Work out the finished part from the listing and answer in its coordinate system (mm). Face numbers are marked on the shaded views. Coordinates: 2 decimals unless noted, no trailing zeros. Loops run counter-clockwise (first coordinate to the right, second up) from the corner with the lowest first, then second, coordinate; pieces in that order, holes last.
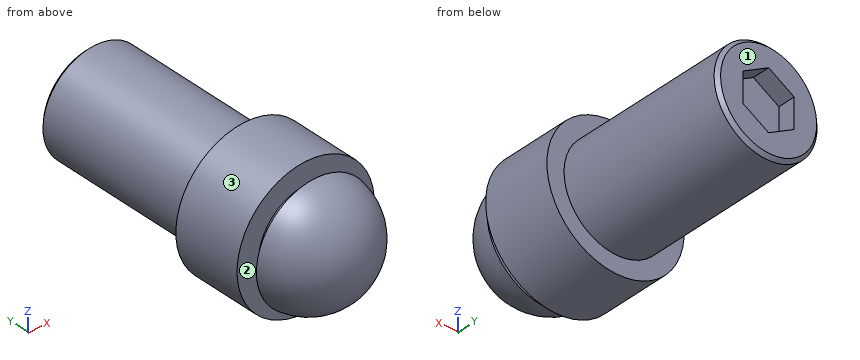
```python
from build123d import *

# Parameters (mm, degrees)
SKETCH1_R           = 1.5
BOSS_EXTRUDE1_DEPTH = 5
SKETCH2_R           = 2
BOSS_EXTRUDE2_DEPTH = 2
CUT_EXTRUDE1_DEPTH  = 0.5
CHAMFER1_SIZE       = 0.1


with BuildPart() as part:
    # Sketch1 → Boss-Extrude1 (new body)
    with BuildSketch(Plane(origin=(0, 0, 0), x_dir=(1, 0, 0), z_dir=(0, 1, 0))):
        with Locations(Location((0, 0, 0), (0, 0, 270))):
            Circle(SKETCH1_R)
    extrude(amount=BOSS_EXTRUDE1_DEPTH)

    # Sketch2 → Boss-Extrude2 (add)
    with BuildSketch(Plane.XZ):
        with Locations(Location((0, 0, 0), (0, 0, 270))):
            Circle(SKETCH2_R)
    extrude(amount=BOSS_EXTRUDE2_DEPTH)

    # Sketch3 → Revolve1 (revolve)
    with BuildSketch(Plane.XY):
        with BuildLine():
            Line((0, -2), (0, -3.798690772))
            ThreePointArc((0, -3.798690772), (1.135010023, -3.368611599), (1.7, -2.294366668))
            Line((1.7, -2.294366668), (1.376675655, -2.294366668))
            Line((1.376675655, -2.294366668), (1.376675655, -2))
            Line((1.376675655, -2), (0, -2))
        make_face()
    revolve(axis=Axis((0, -2, 0), (0, -1, 0)))

    # Sketch4 → Cut-Extrude1 (cut)
    with BuildSketch(Plane(origin=(0, 5, 0), x_dir=(1, 0, 0), z_dir=(0, 1, 0))):
        Polygon((0, 0.860152501), (-0.744913917, 0.430076251), (-0.744913917, -0.430076251), (0, -0.860152501), (0.744913917, -0.430076251), (0.744913917, 0.430076251), align=None)
    extrude(amount=-CUT_EXTRUDE1_DEPTH, mode=Mode.SUBTRACT)

    # Chamfer1
    chamfer1_edges = [part.edges().sort_by_distance(p)[0] for p in [
        (0, 5, -1.5),
    ]]
    chamfer(chamfer1_edges, length=CHAMFER1_SIZE)


solid = part.part
```
1. A cutting plane is placed at A-A, the plane z = 0. Give the vertices of the cut face in (x, y), then the cut area to 3 significant figures.
2. Each of these flat-tipped pins is pushed along its axis until it touches: P1, Ø2, axis at y = 2, z = -1, coming from the -X side; P2, Ø1.5, axis at y = -0.5, z = -1, coming from the +X side; P3, Ø1.5, axis at y = -2.5, z = -1.5, coming from the +X side. Where does it stop, or does it pass through?
3. A cutting plane is placed at C-C, the plane y = 1. Give the vertices of the cut face in (x, z).
4. Straight lines are drawn through the part: probe 1 along Y at (x, z) = (0.95, -1.6); probe 2 along Y at (x, z) = (0, -1.45); probe 3 along X at (y, z) = (1.25, 1.3). For each, find the intervals that lie inside material, in ascending order.
5. A cutting plane is placed at B-B, the plane y = -0.25. Give the vertices of the cut face in (x, z).
6. Determine the mould class of the marked faces 1, 2 and 3 for opening direction Y: released by +Y, released by -Y, zero draft, split by the parting line, or undercut.
Answers below:
1. outline: (-2, -2) - (-1.38, -2) - (-1.38, -2.29) - (-1.7, -2.29) arc R1.71 ccw to (1.7, -2.29) - (1.38, -2.29) - (1.38, -2) - (2, -2) - (2, 0) - (1.5, 0) - (1.5, 4.9) - (1.4, 5) - (0.74, 5) - (0.74, 4.5) - (-0.74, 4.5) - (-0.74, 5) - (-1.4, 5) - (-1.5, 4.9) - (-1.5, 0) - (-2, 0) - close
1. area: 27.0 mm2
2. P1: stops at x = -1.5
2. P2: stops at x = 1.98
2. P3: stops at x = 1.76
3. outline: circle Ø3 at (0, 0)
4. probe 1: y = -2 to 0
4. probe 2: y = -3 to -2.29, -2 to 4.95
4. probe 3: x = -0.75 to 0.75
5. outline: circle Ø4 at (0, 0)
6. face 1: released by +Y
6. face 2: undercut
6. face 3: zero draft
